Source: three-view drawing plus pictorial views. Frame: mm from the lowest corner of the part. Give positions to 0.01 mm unless a question says otherwise; leave off trailing zeros. Loops run counter-clockwise (first coordinate to the right, second up) from the corner with the lowest first, then second, coordinate; pieces in that order, holes last. Notation, with made-up numbers: M -7,-35 L 40,-35 A37 ccw 40,3 Z; hole C 69,29.25 d10. An arc over 180 degrees is marked long. Answer as a JSON object with one key per item and string values. Group by question number.
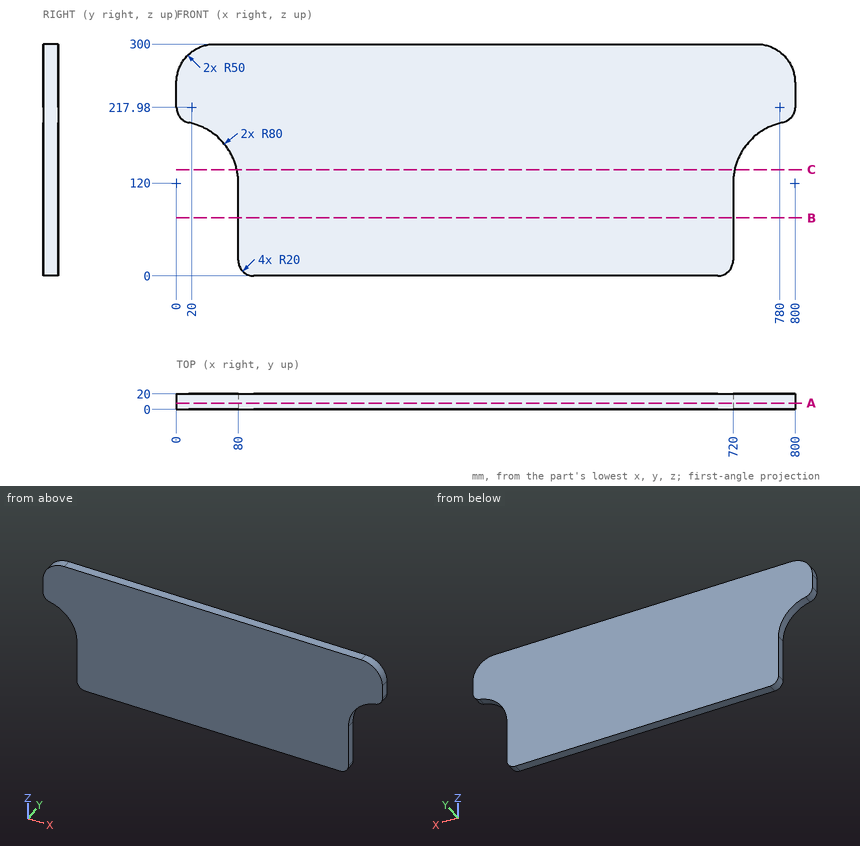
1. Section B-B (z = 75). Output: boundary loops of the cut face in (x, y).
2. Section A-A (y = 8.25). Output: boundary loops of the cut face in (x, z).
3. First-contact query: P1, Ø2, axis at x = 708.5, y = 7, coming from the -Z side; P2, Ø10, axis at y = 5, z = 105.5, coming from the +X side; P3, Ø6, axis at y = 17.5, z = 211.5, coming from the -X side (1 decimal); P4, Ø12, axis at x = 407.5, y = 6.5, coming from the -Z side. Flat tips, straight axial feed; report the tip coordinate or a pass-through.
4. Section C-C (z = 137.5). Output: boundary loops of the cut face in (x, y).
5. Material intervals for L1, parallel to X at y = 3, z = 53; L2, parallel to X at y = 6, z = 215.5 (1 decimal); L3, parallel to Z at x = 702, y = 15.5, sorted ascending.
Geometry results:
{
 "1": {"outline": "M 80,0 L 720,0 L 720,20 L 80,20 Z"},
 "2": {"outline": "M 0,217.98 A20 ccw 16,198.38 A80 cw 80,120 L 80,20 A20 ccw 100,0 L 700,0 A20 ccw 720,20 L 720,120 A80 cw 784,198.38 A20 ccw 800,217.98 L 800,250 A50 ccw 750,300 L 50,300 A50 ccw 0,250 Z"},
 "3": {"P1": "z = 1.46", "P2": "x = 720", "P3": "x = 0.3", "P4": "z = 0"},
 "4": {"outline": "M 78.06,0 L 721.94,0 L 721.94,20 L 78.06,20 Z"},
 "5": {"L1": "80 to 720", "L2": "0.2 to 799.8", "L3": "0.1 to 300"}
}
